Check sheet for the drawn part. Datum: minimum x, y, z corner. Units: mm. A direction names the side the tool comes from. Coordinates: 2 decimals unless noted, no trailing zeros. Write each loop counter-clockwise with the first axis right and the second up, starting at its lowest first coordinate (ties: lowest second). Pieces come first, ordered by that corner, then holes. Notation, with made-up numbers: (42, -20) - (65, -20) arc R22 ccw to (65, -5) - close; hole circle Ø10 at (-25, 19.5). An arc over 180 degrees is marked (long way). Use one line per item in the form item = value. Start each with the question number.
1. Go/stop test with flat-tipped pins: pin 1 Ø1.5 at (x, y) = (1.5, 19.5) entering from +Z; pin 2 Ø1.5 at (x, z) = (3.5, 3.5) entering from +Y; pin 3 Ø2 at (y, z) = (9.5, 1.5) entering from +X. Record where each tip stops, or that it passes through.
2. Scan lines: line 1 along Y through (x, z) = (5, 5.5); line 2 along Y through (x, z) = (3.25, 4); line 3 along X through (y, z) = (1, 4.25) (1 decimal). Record each from-to range of solid material in increasing order.
3. Tool access check on the marked faces 1, 2 and 3. Record the directions out of +Z, -Z, +X, -X, +Y, -Y that give a thin tool (end or side, any length) a straight path to the whole face; none if there is none.
4. Cross-section at A-A on y = 17.5. Record the boundary of the cut face in (x, z), then the cut area to 3 significant figures.
5. Draft check along Z on the marked faces 4, 5 and 6. Enter one of: +Z half, -Z half, draft (parallel to the pull), parting line (faces both ways), or undercut.
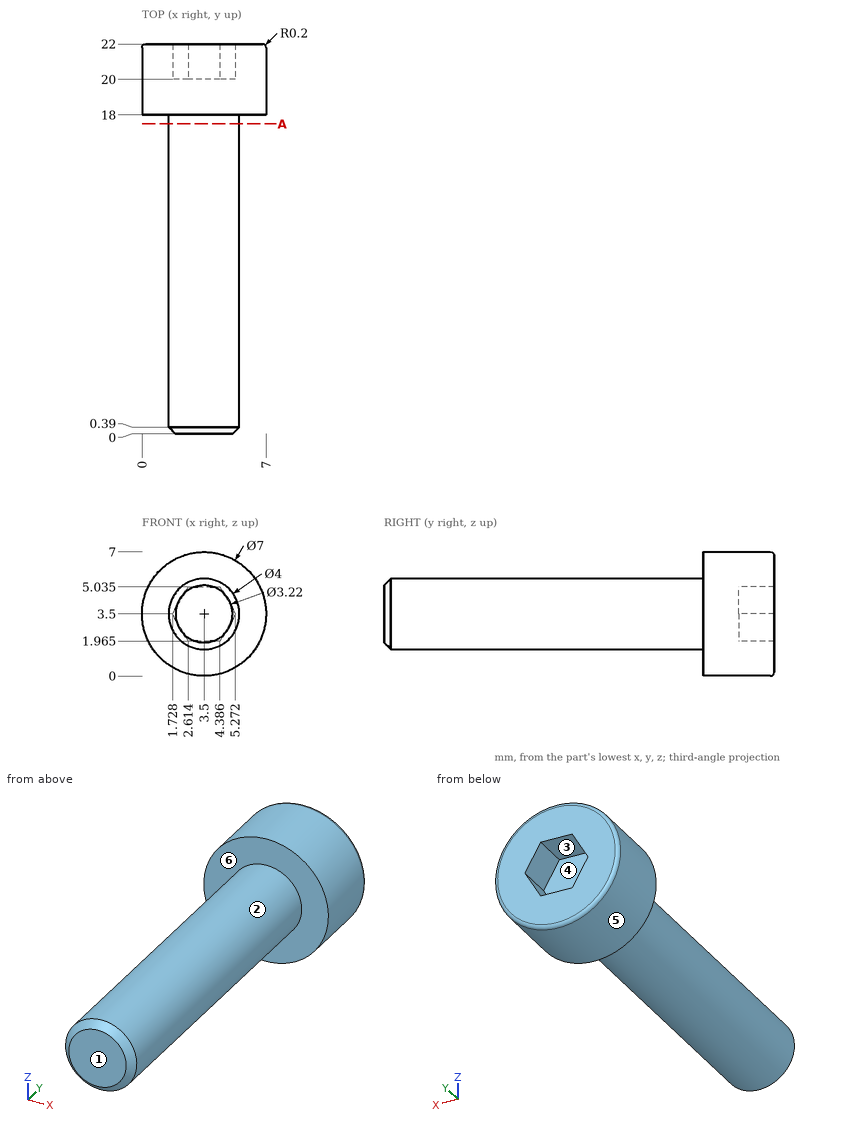
Final values:
q1.pin_1 = 6.77
q1.pin_2 = 20
q1.pin_3 = 5.23
q2.line_1 = 18 to 22
q2.line_2 = 0 to 20
q2.line_3 = 1.6 to 5.4
q3.face_1 = +Z, -Z, +X, -X, -Y
q3.face_2 = -Y
q3.face_3 = +Y
q4.outline = circle Ø4 at (3.5, 3.5)
q4.area = 12.6 mm²
q5.face_4 = undercut
q5.face_5 = parting line
q5.face_6 = draft
